```python
from build123d import *

# Parameters (mm, degrees)
BOSS_EXTRUDE1_DEPTH = 8
SKETCH3_R           = 8
CUT_EXTRUDE1_DEPTH  = 8
CUT_EXTRUDE2_DEPTH  = 115.30458075
FILLET1_R           = 5


with BuildPart() as part:
    # Sketch2 → Boss-Extrude1 (new body)
    with BuildSketch(Plane.XY):
        with BuildLine():
            Line((0, 0), (0, 65))
            Line((0, 65), (12.679491924, 86.961524227))
            ThreePointArc((12.679491924, 86.961524227), (30, 96.961524227), (47.320508076, 86.961524227))
            Line((47.320508076, 86.961524227), (60, 65))
            Line((60, 65), (60, 0))
            Line((60, 0), (0, 0))
        make_face()
    extrude(amount=BOSS_EXTRUDE1_DEPTH)

    # Sketch3 → Cut-Extrude1 (cut)
    with BuildSketch(Plane.XY.offset(8)):
        with Locations((30, 80)):
            Circle(SKETCH3_R)
    extrude(amount=-CUT_EXTRUDE1_DEPTH, mode=Mode.SUBTRACT)

    # Sketch4 → Cut-Extrude2 (cut, through all)
    with BuildSketch(Plane.XY.offset(8)):
        with BuildLine():
            Line((10.5, 12), (10.5, 42))
            ThreePointArc((10.5, 42), (15, 46.5), (19.5, 42))
            Line((19.5, 42), (19.5, 12))
            ThreePointArc((19.5, 12), (15, 7.5), (10.5, 12))
        make_face()
        with BuildLine():
            Line((49.5, 12), (49.5, 42))
            ThreePointArc((49.5, 42), (45, 46.5), (40.5, 42))
            Line((40.5, 42), (40.5, 12))
            ThreePointArc((40.5, 12), (45, 7.5), (49.5, 12))
        make_face()
    extrude(amount=-CUT_EXTRUDE2_DEPTH, mode=Mode.SUBTRACT)

    # Fillet1
    fillet1_edges = [part.edges().sort_by_distance(p)[0] for p in [
        (0, 65, 4),
        (60, 65, 4),
    ]]
    fillet(fillet1_edges, radius=FILLET1_R)


solid = part.part
```
Verification items for the finished model (mm, model axes). A direction names the side the tool comes from. Round coordinates to 2 decimals unless told otherwise and drop trailing zeros. Loops run counter-clockwise (first coordinate to the right, second up) from the corner with the lowest first, then second, coordinate; pieces in that order, holes last. Notation, with made-up numbers: (79.25, 31.25) -> (132.25, 31.25) arc R17 ccw to (132.25, 64.25) -> close; hole circle Ø7 at (87, 31). An arc over 180 degrees is marked (long way). Answer as a JSON object with one key per item and string values.
Q1. Access from +Z, -Z, +X, -X, +Y, -Y to the whole of each face (thin tool, end or side, straight path). Record for faces 4 (the cylindrical face through (14.9, 46.5, 4.1)), 5 (the flat face through (30, 49, 0)).
Data:
{"face 4": "+Z, -Z", "face 5": "-Z, +X, -X, +Y, -Y"}
Q2. Scan lines: line 1 (X direction, y = 24, z = 2.25); line 2 (X direction, y = 11, z = 3.25); line 3 (X direction, y = 75.5, z = 6.5). Record each from-to range of solid material in increasing order. Write a range as from..to.
Data:
{"line 1": "x = 0..10.5, 19.5..40.5, 49.5..60", "line 2": "x = 0..10.61, 19.39..40.61, 49.39..60", "line 3": "x = 6.06..23.39, 36.61..53.94"}
Q3. Section check C-C (z = 7). Record the boundary of the cut face in (x, y), then the cut area to 3 significant figures.
Data:
{"outline": "(0, 0) -> (60, 0) -> (60, 63.66) arc R5 ccw to (59.33, 66.16) -> (47.32, 86.96) arc R20 ccw to (12.68, 86.96) -> (0.67, 66.16) arc R5 ccw to (0, 63.66) -> close; hole (10.5, 12) arc R4.5 ccw to (19.5, 12) -> (19.5, 42) arc R4.5 ccw to (10.5, 42) -> close; hole circle Ø16 at (30, 80); hole (40.5, 12) arc R4.5 ccw to (49.5, 12) -> (49.5, 42) arc R4.5 ccw to (40.5, 42) -> close", "area": "4,320 mm2"}
Q4. Draft check along X on faces 1 (the cylindrical face through (0.166, 64.937, 4.056)), 2 (the flat face through (30, 0, 4)), 3 (the flat face through (40.5, 27, 4)). Enter one of: pulls with the +X half, pulls with the -X half, needs draft (parallel to the pull), parting line crosses it, or undercut.
Data:
{"face 1": "pulls with the -X half", "face 2": "needs draft", "face 3": "undercut"}
Q5. Section check A-A (x = 30). Record the boundary of the cut face in (y, z), then the cut area to 3 significant figures.
Data:
{"outline": "(0, 0) -> (72, 0) -> (72, 8) -> (0, 8) -> close; (88, 0) -> (96.96, 0) -> (96.96, 8) -> (88, 8) -> close", "area": "648 mm2"}
Q6. Section check B-B (y = 20). Record the boundary of the cut face in (x, z), then the cut area to 3 significant figures.
Data:
{"outline": "(0, 0) -> (10.5, 0) -> (10.5, 8) -> (0, 8) -> close; (19.5, 0) -> (40.5, 0) -> (40.5, 8) -> (19.5, 8) -> close; (49.5, 0) -> (60, 0) -> (60, 8) -> (49.5, 8) -> close", "area": "336 mm2"}
Q7. Section check D-D (y = 82). Record the boundary of the cut face in (x, z), then the cut area to 3 significant figures.
Data:
{"outline": "(9.81, 0) -> (22.25, 0) -> (22.25, 8) -> (9.81, 8) -> close; (37.75, 0) -> (50.19, 0) -> (50.19, 8) -> (37.75, 8) -> close", "area": "199 mm2"}
